Design review of the part built by this model. Coordinates are the model's own, in mm. A direction names the side the tool comes from. Coordinates: 2 decimals unless noted, no trailing zeros. Order: outer loops, then holes, each group sorted by start corner. A loop starts at its lowest first (then second) coordinate and runs counter-clockwise, first axis right, second up.
from build123d import *

# Parameters (mm, degrees)
BASE_PLATE_SKETCH_W        = 90
BASE_PLATE_SKETCH_H        = 135
BASE_PLATE_DEPTH           = 12
MOUNTING_HOLES_SKETCH_R    = 8
MOUNTING_HOLES_2X_16_DEPTH = 22
CLEVIS_ARM_SKETCH_R        = 20
CLEVIS_ARM_SKETCH_R_2      = 8
CLEVIS_ARM_DEPTH           = 22.5
CLEVIS_SLOT_DEPTH          = 162.074413963
CLEVIS_SLOT_DEPTH_BACK     = 162.074413963
CLEVIS_SLOT_SKETCH_W       = 40
CLEVIS_SLOT_SKETCH_H       = 25
PIN_HOLE_DEPTH             = 165.465701085
PIN_HOLE_DEPTH_BACK        = 165.465701085
PIN_HOLE_SKETCH_W          = 94.002676874
PIN_HOLE_SKETCH_H          = 25
LUG_BOSS_1_SKETCH_R        = 20
LUG_BOSS_1_SKETCH_R_2      = 8
LUG_BOSS_1_40_DEPTH        = 4
LUG_START                  = 4
LUG_BOSS_2_SKETCH_R        = 20
LUG_BOSS_2_SKETCH_R_2      = 8
LUG_BOSS_2_40_DEPTH        = 4
LUG_BOSS_3_SKETCH_R        = 20
LUG_BOSS_3_SKETCH_R_2      = 8
LUG_BOSS_3_40_DEPTH        = 4
LUG_BOSS_4_SKETCH_R        = 20
LUG_BOSS_4_SKETCH_R_2      = 8
LUG_BOSS_4_40_DEPTH        = 4


with BuildPart() as part:
    # Base Plate Sketch → Base Plate (new body)
    with BuildSketch(Plane.XY):
        Rectangle(BASE_PLATE_SKETCH_W, BASE_PLATE_SKETCH_H)
    extrude(amount=BASE_PLATE_DEPTH)

    # Mounting Holes Sketch → Mounting Holes 2xØ16 (cut)
    with BuildSketch(Plane.XY.offset(12)):
        with Locations((5, -45.5)):
            Circle(MOUNTING_HOLES_SKETCH_R)
        with Locations((5, 45.5)):
            Circle(MOUNTING_HOLES_SKETCH_R)
    extrude(amount=-MOUNTING_HOLES_2X_16_DEPTH, mode=Mode.SUBTRACT)

    # Clevis Arm Sketch → Clevis Arm (add, symmetric)
    # profile 1 of 2: a face of its own
    with BuildSketch(Plane(origin=(0, 0, 0), x_dir=(1, 0, 0), z_dir=(0, 1, 0))):
        with BuildLine():
            Line((-120.672374095, -12), (-45, -12))
            Line((-45, -12), (-45, 0))
            Line((-45, 0), (45, 0))
            Line((45, 0), (-3.672374095, 40))
            Line((-3.672374095, 40), (-122.695594955, 27.897401271))
            ThreePointArc((-122.695594955, 27.897401271), (-107.264622926, 22.84022266), (-100.672374095, 8))
            ThreePointArc((-100.672374095, 8), (-106.530238471, -6.142135624), (-120.672374095, -12))
        make_face()
    # profile 2 of 2: a face of its own
    with BuildSketch(Plane(origin=(0, 0, 0), x_dir=(1, 0, 0), z_dir=(0, 1, 0))):
        with Locations((-120.672374095, 8)):
            Circle(CLEVIS_ARM_SKETCH_R)
        with Locations(Location((-120.672374095, 8, 0), (0, 0, 90))):
            Circle(CLEVIS_ARM_SKETCH_R_2, mode=Mode.SUBTRACT)
    extrude(amount=CLEVIS_ARM_DEPTH, both=True)

    # Clevis Slot Sketch → Clevis Slot (cut, two sides: drawn at the far end of the back side and taken through both)
    with BuildSketch(Plane(origin=(0, 0, 0), x_dir=(0, 0, -1), z_dir=(1, 0, 0)).offset(-CLEVIS_SLOT_DEPTH_BACK)):
        with Locations((20, 0)):
            Rectangle(CLEVIS_SLOT_SKETCH_W, CLEVIS_SLOT_SKETCH_H)
    extrude(amount=CLEVIS_SLOT_DEPTH + CLEVIS_SLOT_DEPTH_BACK, mode=Mode.SUBTRACT)

    # Pin Hole Sketch → Pin Hole (cut, two sides: drawn at the far end of the back side and taken through both)
    with BuildSketch(Plane.XY.offset(12).offset(-PIN_HOLE_DEPTH_BACK)):
        with Locations((-92.001338437, 0)):
            Rectangle(PIN_HOLE_SKETCH_W, PIN_HOLE_SKETCH_H)
    extrude(amount=PIN_HOLE_DEPTH + PIN_HOLE_DEPTH_BACK, mode=Mode.SUBTRACT)

    # Lug Boss 1 Sketch → Lug Boss 1 Ø40 (add)
    with BuildSketch(Plane.XZ.offset(22.5)):
        with Locations(Location((-120.672374095, -8, 0), (0, 0, 270))):
            Circle(LUG_BOSS_1_SKETCH_R)
        with Locations(Location((-120.672374095, -8, 0), (0, 0, 270))):
            Circle(LUG_BOSS_1_SKETCH_R_2, mode=Mode.SUBTRACT)
    extrude(amount=LUG_BOSS_1_40_DEPTH)

    # Lug Boss 2 Sketch → Lug Boss 2 Ø40 (add)
    with BuildSketch(Plane(origin=(0, -12.5, 0), x_dir=(1, 0, 0), z_dir=(0, 1, 0)).offset(LUG_START)):
        with Locations(Location((-120.672374095, 8, 0), (0, 0, 90))):
            Circle(LUG_BOSS_2_SKETCH_R)
        with Locations(Location((-120.672374095, 8, 0), (0, 0, 90))):
            Circle(LUG_BOSS_2_SKETCH_R_2, mode=Mode.SUBTRACT)
    extrude(amount=-LUG_BOSS_2_40_DEPTH)

    # Lug Boss 3 Sketch → Lug Boss 3 Ø40 (add)
    with BuildSketch(Plane(origin=(0, 22.5, 0), x_dir=(1, 0, 0), z_dir=(0, 1, 0)).offset(LUG_START)):
        with Locations(Location((-120.672374095, 8, 0), (0, 0, 270))):
            Circle(LUG_BOSS_3_SKETCH_R)
        with Locations(Location((-120.672374095, 8, 0), (0, 0, 90))):
            Circle(LUG_BOSS_3_SKETCH_R_2, mode=Mode.SUBTRACT)
    extrude(amount=-LUG_BOSS_3_40_DEPTH)

    # Lug Boss 4 Sketch → Lug Boss 4 Ø40 (add)
    with BuildSketch(Plane.XZ.offset(-12.5)):
        with Locations(Location((-120.672374095, -8, 0), (0, 0, 270))):
            Circle(LUG_BOSS_4_SKETCH_R)
        with Locations(Location((-120.672374095, -8, 0), (0, 0, 270))):
            Circle(LUG_BOSS_4_SKETCH_R_2, mode=Mode.SUBTRACT)
    extrude(amount=LUG_BOSS_4_40_DEPTH)


solid = part.part
1. Add section D-D (x = -109.5). Give the boundary of the cut face in (y, z), and give its area (3 significant figures).
2. Add section C-C (z = 9). Give the boundary of the cut face in (x, y).
3. For faces 1 (the cylindrical face through (-140.502, -17.374, -5.396)), 2 (the flat face through (-112, -8.5, -8)), 3 (the flat face through (-11, 45, 0)), list the 3-axis set-ups (+Z, -Z, +X, -X, +Y, -Y) from which the entire face can be reached by the end or side of a thin tool; tool diameter is ignored.
4. To check wall thickness, follow line 1 (Y direction, x = 5, z = 2); line 2 (Y direction, x = 25.5, z = -8.5); line 3 (X direction, y = 45, z = 5). State the ranges of each line that lie inside material, in increasing order.
5. Add section B-B (x = 5). Give the boundary of the cut face in (y, z).
6. Add section A-A (y = -45.5). Give the boundary of the cut face in (x, z), and give its area (3 significant figures).
7. Mouldability with a two-part tool opening along X and no side actions: class faces 4 (the cylindrical face through (9.301, -38.754, 6.084)), 5 (the flat face through (-120, 26.5, 1)), 6 (the flat face through (-62.351, -17.43, -34.033)) as pulls with the +X half, pulls with the -X half, needs draft (parallel to the pull), parting line crosses it, or undercut.
8. Insertion check: pin 1 (9.5 mm diameter, centred on x = -120.67, z = -8, fed in from +Y); pin 2 (20 mm diameter, centred on x = -127.5, z = -1.5, fed in from -Y); pin 3 (10 mm diameter, centred on x = -13, z = -33.5, fed in from +Y); pin 4 (4 mm diameter, centred on y = 7, z = -24, fed in from -X). Each pin has a flat end and moves straight along its axis. Give the tip position at first contact, or say it passes through.
Solution:
1. outline: (-26.5, -24.59) - (-22.5, -24.59) - (-22.5, -29.24) - (-12.5, -29.24) - (-12.5, -24.59) - (-8.5, -24.59) - (-8.5, 8.59) - (-12.5, 8.59) - (-12.5, 12) - (-22.5, 12) - (-22.5, 8.59) - (-26.5, 8.59) - close; (8.5, -24.59) - (12.5, -24.59) - (12.5, -29.24) - (22.5, -29.24) - (22.5, -24.59) - (26.5, -24.59) - (26.5, 8.59) - (22.5, 8.59) - (22.5, 12) - (12.5, 12) - (12.5, 8.59) - (8.5, 8.59) - close
1. area: 1,360 mm2
2. outline: (-131.21, -26.5) - (-110.14, -26.5) - (-110.14, -22.5) - (-45, -22.5) - (-45, -67.5) - (45, -67.5) - (45, 67.5) - (-45, 67.5) - (-45, 22.5) - (-110.14, 22.5) - (-110.14, 26.5) - (-131.21, 26.5) - (-131.21, 8.5) - (-110.14, 8.5) - (-110.14, 12.5) - (-45, 12.5) - (-45, -12.5) - (-110.14, -12.5) - (-110.14, -8.5) - (-131.21, -8.5) - close; hole circle Ø16 at (5, -45.5); hole circle Ø16 at (5, 45.5)
3. face 1: none
3. face 2: +Z, -Z, -X
3. face 3: -Z, +X, +Y
4. line 1: y = -67.5 to -53.5, -37.5 to 37.5, 53.5 to 67.5
4. line 2: y = -22.5 to -12.5, 12.5 to 22.5
4. line 3: x = -45 to -2.98, 12.98 to 45
5. outline: (-67.5, 0) - (-53.5, 0) - (-53.5, 12) - (-67.5, 12) - close; (-37.5, 0) - (-22.5, 0) - (-22.5, -32.87) - (-12.5, -32.87) - (-12.5, 0) - (12.5, 0) - (12.5, -32.87) - (22.5, -32.87) - (22.5, 0) - (37.5, 0) - (37.5, 12) - (-37.5, 12) - close; (53.5, 0) - (67.5, 0) - (67.5, 12) - (53.5, 12) - close
6. outline: (-45, 0) - (-3, 0) - (-3, 12) - (-45, 12) - close; (13, 0) - (45, 0) - (45, 12) - (13, 12) - close
6. area: 888 mm2
7. face 4: undercut
7. face 5: needs draft
7. face 6: pulls with the -X half
8. pin 1: passes through
8. pin 2: stops at y = -26.5
8. pin 3: stops at y = 22.5
8. pin 4: stops at x = -134.26
